```python
from build123d import *

# Parameters (mm, degrees)
LINK_PLATE_20MM_DEPTH       = 20
CENTRE_OPENING_SKETCH_R     = 67.8
CENTRE_OPENING_135_6_DEPTH  = 20
ANNULAR_WEB_SKETCH_R        = 67.8
ANNULAR_WEB_SKETCH_R_2      = 40
ANNULAR_WEB_80X_135_6_DEPTH = 10


with BuildPart() as part:
    # Link Plate Outline Sketch → Link Plate 20mm (new body)
    with BuildSketch(Plane.XY):
        with BuildLine():
            Line((-38.729833462, 10), (-22.912878475, 10))
            ThreePointArc((-22.912878475, 10), (25, 0), (-22.912878475, -10))
            Line((-22.912878475, -10), (-38.729833462, -10))
            ThreePointArc((-38.729833462, -10), (-14.281675999, -37.363534772), (22.185185185, -33.283893377))
            ThreePointArc((22.185185185, -33.283893377), (58.387841465, -25.611592996), (89.95, -44.933256058))
            ThreePointArc((89.95, -44.933256058), (150, -75), (210.05, -44.933256058))
            ThreePointArc((210.05, -44.933256058), (241.612158535, -25.611592996), (277.814814815, -33.283893377))
            ThreePointArc((277.814814815, -33.283893377), (314.281675999, -37.363534772), (338.729833462, -10))
            Line((338.729833462, -10), (322.912878475, -10))
            ThreePointArc((322.912878475, -10), (275, 0), (322.912878475, 10))
            Line((322.912878475, 10), (338.729833462, 10))
            ThreePointArc((338.729833462, 10), (314.281675999, 37.363534772), (277.814814815, 33.283893377))
            ThreePointArc((277.814814815, 33.283893377), (241.612158535, 25.611592996), (210.05, 44.933256058))
            ThreePointArc((210.05, 44.933256058), (150, 75), (89.95, 44.933256058))
            ThreePointArc((89.95, 44.933256058), (58.387841465, 25.611592996), (22.185185185, 33.283893377))
            ThreePointArc((22.185185185, 33.283893377), (-14.281675999, 37.363534772), (-38.729833462, 10))
        make_face()
    extrude(amount=LINK_PLATE_20MM_DEPTH)

    # Centre Opening Sketch → Centre Opening Ø135.6 (cut)
    with BuildSketch(Plane.XY.offset(20)):
        with Locations((150, 0)):
            Circle(CENTRE_OPENING_SKETCH_R)
    extrude(amount=-CENTRE_OPENING_135_6_DEPTH, mode=Mode.SUBTRACT)

    # Annular Web Sketch → Annular Web Ø80xØ135.6 (add)
    with BuildSketch(Plane.XY.offset(10)):
        with Locations((150, 0)):
            Circle(ANNULAR_WEB_SKETCH_R)
        with Locations((150, 0)):
            Circle(ANNULAR_WEB_SKETCH_R_2, mode=Mode.SUBTRACT)
    extrude(amount=-ANNULAR_WEB_80X_135_6_DEPTH)


solid = part.part
```
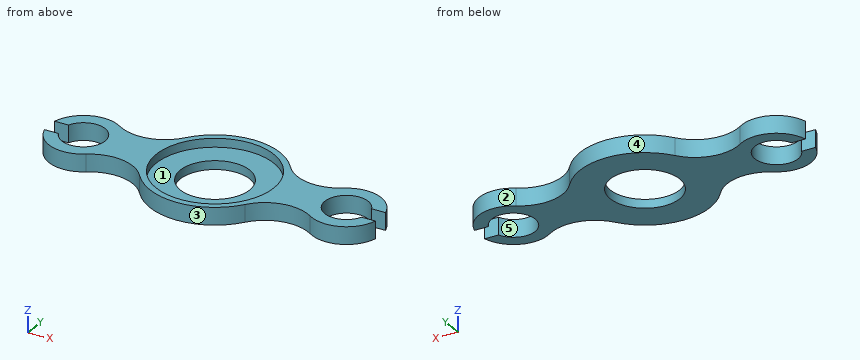
The listing builds one solid part. Answer for the finished solid, in the listing's coordinates (mm). Face numbers are marked on the shaded views. A direction names the side the tool comes from. Give positions to 0.01 mm unless a question says otherwise; leave off trailing zeros. Order: outer loops, then holes, each group sorted by start corner. A loop starts at its lowest first (then second) coordinate and runs counter-clockwise, first axis right, second up. Notation, with made-up numbers: (-5.5, 11) -> (8.5, 11) arc R16 ccw to (8.5, 22) -> close; hole circle Ø8 at (23, 6.5). An arc over 180 degrees is marked (long way). Write each question's results on one line, items separated by ' | '.
Q1. The part is cut by section B-B, the plane y = -5.5. Give the vertices of the cut face in (x, z), and give its area (3 significant figures).
Checked values:
outline: (24.39, 0) -> (110.38, 0) -> (110.38, 10) -> (82.42, 10) -> (82.42, 20) -> (24.39, 20) -> close; (189.62, 0) -> (275.61, 0) -> (275.61, 20) -> (217.58, 20) -> (217.58, 10) -> (189.62, 10) -> close | area: 2,880 mm^2
Q2. Each of these flat-tipped pins is pushed along its axis until it touches: P1, Ø4.5, axis at x = -30.5, z = 12.5, coming from the -Y side; P2, Ø2, axis at x = 183.5, z = 11, coming from the +Y side; P3, Ø6, axis at x = 134, z = 15, coming from the +Y side. Where does it stop, or does it pass through?
Checked values:
P1: stops at y = -28.32 | P2: stops at y = 67.59 | P3: stops at y = 73.86
Q3. Determine the mould class of the marked faces 3, 4 and 5 for opening direction Y: pulls with the +Y half, pulls with the -Y half, needs draft (parallel to the pull), parting line crosses it, or undercut.
Checked values:
face 3: pulls with the -Y half | face 4: pulls with the +Y half | face 5: undercut
Q4. The part is cut by section D-D, the plane x = 150. Give the vertices of the cut face in (y, z), and give its area (3 significant figures).
Checked values:
outline: (-75, 0) -> (-40, 0) -> (-40, 10) -> (-67.8, 10) -> (-67.8, 20) -> (-75, 20) -> close; (40, 0) -> (75, 0) -> (75, 20) -> (67.8, 20) -> (67.8, 10) -> (40, 10) -> close | area: 844 mm^2
Q5. Which of the six approach directions +Z, -Z, +X, -X, +Y, -Y give full straight-line access (tool end or side, diameter ignored) to the marked faces 1 and 2?
Checked values:
face 1: +Z | face 2: +Z, -Z, +Y
Q6. The part is cut by section C-C, the plane z = 13.75. Give the vertices of the cut face in (x, y).
Checked values:
outline: (-38.73, -10) arc R40 ccw to (22.19, -33.28) arc R50 cw to (89.95, -44.93) arc R75 ccw to (210.05, -44.93) arc R50 cw to (277.81, -33.28) arc R40 ccw to (338.73, -10) -> (322.91, -10) arc R25 cw (long way) to (322.91, 10) -> (338.73, 10) arc R40 ccw to (277.81, 33.28) arc R50 cw to (210.05, 44.93) arc R75 ccw to (89.95, 44.93) arc R50 cw to (22.19, 33.28) arc R40 ccw to (-38.73, 10) -> (-22.91, 10) arc R25 cw (long way) to (-22.91, -10) -> close; hole circle Ø135.6 at (150, 0)
Q7. Straight lines are drawn through the part: probe 1 along X at (y, z) = (18, 8.75); probe 2 along Y at (x, z) = (0, 12.25); probe 3 along Y at (x, z) = (315, 5.5). For each, find the intervals that lie inside material, in ascending order. Write a range as from..to.
Checked values:
probe 1: x = -35.72..-17.35, 17.35..114.28, 185.72..282.65, 317.35..335.72 | probe 2: y = -40..-25, 25..40 | probe 3: y = -37.08..-20, 20..37.08
Q8. The part is cut by section A-A, the plane x = 0. Give the vertices of the cut face in (y, z).
Checked values:
outline: (-40, 0) -> (-25, 0) -> (-25, 20) -> (-40, 20) -> close; (25, 0) -> (40, 0) -> (40, 20) -> (25, 20) -> close
